Could you check a few things on this model? Use its own coordinates, in mm. A direction names the side the tool comes from. Give positions to 0.01 mm unless a question says otherwise; leave off trailing zeros. Loops run counter-clockwise (first coordinate to the right, second up) from the corner with the lowest first, then second, coordinate; pieces in that order, holes last. Notation, with made-up numbers: (82.25, 30.5) -> (135.25, 30.5) arc R35 cw to (135.25, 68.5) -> close; hole circle Ø4 at (8.5, 20.25). An arc over 180 degrees is marked (long way). Put each result on its own line as item: value.
```python
from build123d import *

# Parameters (mm, degrees)
SKETCH_1_W      = 18
SKETCH_1_H      = 8
EXTRUDE_1_DEPTH = 10
SKETCH_2_W      = 18
SKETCH_2_H      = 2
EXTRUDE_2_DEPTH = 20


with BuildPart() as part:
    # 草图1 → 凸台-拉伸1 (new body)
    with BuildSketch(Plane.XY):
        Rectangle(SKETCH_1_W, SKETCH_1_H)
    extrude(amount=EXTRUDE_1_DEPTH)

    # 草图2 → 凸台-拉伸2 (add)
    with BuildSketch(Plane.XY.offset(10)):
        with Locations((0, 3)):
            Rectangle(SKETCH_2_W, SKETCH_2_H)
    extrude(amount=EXTRUDE_2_DEPTH)

    # 草图3 → M3 螺纹孔1 (revolve, cut)
    with BuildSketch(Plane.YZ.offset(5)):
        Polygon((0, 0), (0, 7.251075774), (1.25, 6.5), (1.25, 0.275), (1.525, 0), align=None)
    hole_wizard_m3_1 = revolve(axis=Axis((5, 0, -6.35), (0, 0, 1)), mode=Mode.SUBTRACT)

    # 镜向1: M3 螺纹孔1 across plane
    add(hole_wizard_m3_1.mirror(Plane(origin=(0, 0, 0), x_dir=(0, 0, 1), z_dir=(1, 0, 0))), mode=Mode.SUBTRACT)


solid = part.part
```
1. If we section it at A-A (z = 4.5): List the corners of the cut face in (x, y) for me.
Recorded:
outline: (-9, -4) -> (9, -4) -> (9, 4) -> (-9, 4) -> close; hole circle Ø2.5 at (-5, 0); hole circle Ø2.5 at (5, 0)
2. If we section it at D-D (z = 14): List the corners of the cut face in (x, y) for me, then the cut area to 3 significant figures.
Recorded:
outline: (-9, 2) -> (9, 2) -> (9, 4) -> (-9, 4) -> close
area: 36.0 mm^2
3. I'm going to push flat-ended pins straight in: pin 1 (4 mm diameter, centred on x = -6, z = 13.5, fed in from -Y); pin 2 (3 mm diameter, centred on x = -1, y = -1, fed in from +Z). Where does each tip first touch, or does it pass through?
Recorded:
pin 1: stops at y = 2
pin 2: stops at z = 10
4. I need wall thicknesses on line 1 (X direction, y = 0, z = 2.75); line 2 (Y direction, x = 5, z = 5.25); line 3 (Y direction, x = -3.5, z = 15.5). Which ranges of each line are inside material? Lowest first, please.
Recorded:
line 1: x = -9 to -6.25, -3.75 to 3.75, 6.25 to 9
line 2: y = -4 to -1.25, 1.25 to 4
line 3: y = 2 to 4
5. For faces 4 (the face through (0, 0, 0)), 5 (the face through (6.22, -0.27, 3.34)), 6 (the face through (0, 2, 20)), which set-ups out of +Z, -Z, +X, -X, +Y, -Y let a thin tool reach every point of the face, with its end or its side?
Recorded:
face 4: -Z, +X, -X, +Y, -Y
face 5: -Z
face 6: +Z, +X, -X, -Y
6. If we section it at B-B (x = -2.5): List the corners of the cut face in (y, z) for me, then the cut area to 3 significant figures.
Recorded:
outline: (-4, 0) -> (4, 0) -> (4, 30) -> (2, 30) -> (2, 10) -> (-4, 10) -> close
area: 120 mm^2
7. If we section it at C-C (y = -2.5): List the corners of the cut face in (x, z) for me.
Recorded:
outline: (-9, 0) -> (9, 0) -> (9, 10) -> (-9, 10) -> close
8. Thinking about a two-plate mould opening in Y: for faces 1 (the face through (4.82, 0.12, 7.12)), 2 (the face through (0, -4, 5)), 3 (the face through (9, 1, 8)), which applies, pulls with the +Y half, pulls with the -Y half, needs draft (parallel to the pull), parting line crosses it, or undercut?
Recorded:
face 1: undercut
face 2: pulls with the -Y half
face 3: needs draft
